For this review, take the finished solid that the model builds, in its own axes (mm). Give positions to 0.01 mm unless a question says otherwise; leave off trailing zeros. Write each loop counter-clockwise with the first axis right and the second up, starting at its lowest first coordinate (ties: lowest second). Pieces come first, ordered by that corner, then holes. Notation, with made-up numbers: M -12,-6 L 18,-6 A11 cw 18,13 Z; hole C -13,-8.75 d3. An arc over 180 degrees is marked long. Write item = value, one per line.
```python
from build123d import *

# Parameters (mm, degrees)
SKETCH_1_W            = 250
SKETCH_1_H            = 80
EXTRUDE_1_DEPTH       = 10
HOLE_WIZARD_9_0_9_1_D = 9
CHAMFER_1_SIZE        = 3
HOLE_WIZARD_M8_1_D    = 6.8
HOLE_WIZARD_M4_1_D    = 3.3


with BuildPart() as part:
    # 草图1 → 凸台-拉伸1 (new body)
    with BuildSketch(Plane.XY):
        with Locations((0, 40)):
            Rectangle(SKETCH_1_W, SKETCH_1_H)
    extrude(amount=EXTRUDE_1_DEPTH)

    # Ø9.0 (9) 直径孔1 (through all)
    with Locations(Plane.XY.offset(10)):
        with Locations((115, 20), (115, 60)):
            hole_wizard_9_0_9_1 = Hole(HOLE_WIZARD_9_0_9_1_D / 2)

    # 镜向1: Ø9.0 (9) 直径孔1 across plane
    add(hole_wizard_9_0_9_1.mirror(Plane(origin=(0, 0, 0), x_dir=(0, 0, 1), z_dir=(1, 0, 0))), mode=Mode.SUBTRACT)

    # 倒角1
    chamfer_1_edges = [part.edges().sort_by_distance(p)[0] for p in [
        (-125, 80, 5),
        (125, 80, 5),
        (125, 0, 5),
        (-125, 0, 5),
    ]]
    chamfer(chamfer_1_edges, length=CHAMFER_1_SIZE)

    # M8 螺纹孔1 (through all)
    with Locations(Plane.XY.offset(10)):
        with Locations((70.5, 60), (70.5, 20)):
            hole_wizard_m8_1 = Hole(HOLE_WIZARD_M8_1_D / 2)

    # 镜向2: M8 螺纹孔1 across plane
    add(hole_wizard_m8_1.mirror(Plane(origin=(0, 0, 0), x_dir=(0, 0, 1), z_dir=(1, 0, 0))), mode=Mode.SUBTRACT)

    # M4 螺纹孔1 (through all)
    with Locations(Plane.XY.offset(10)):
        with Locations((-94.121851999, 75), (-94.121851999, 5)):
            hole_wizard_m4_1 = Hole(HOLE_WIZARD_M4_1_D / 2)

    # 镜向3: M4 螺纹孔1 across plane
    add(hole_wizard_m4_1.mirror(Plane.ZY), mode=Mode.SUBTRACT)


solid = part.part
```
1. We need section C-C, the plane x = 115. Write out the cut boundary in (y, z), then the cut area to 3 significant figures.
Responses:
outline = M 0,0 L 15.5,0 L 15.5,10 L 0,10 Z; M 24.5,0 L 55.5,0 L 55.5,10 L 24.5,10 Z; M 64.5,0 L 80,0 L 80,10 L 64.5,10 Z
area = 620 mm2
2. We need section A-A, the plane x = -70.5. Write out the cut boundary in (y, z), then the cut area to 3 significant figures.
Responses:
outline = M 0,0 L 16.6,0 L 16.6,10 L 0,10 Z; M 23.4,0 L 56.6,0 L 56.6,10 L 23.4,10 Z; M 63.4,0 L 80,0 L 80,10 L 63.4,10 Z
area = 664 mm2
3. Insertion check: P1, Ø7, axis at x = -115, y = 20, coming from the -Z side. The pin has a flat end and moves straight along its axis. Give the tip position at first contact, or say it passes through.
Responses:
P1 = through
4. The part is to be moulded in two halves that separate along Y. For faces 1 (the face through (-125, 39, 5)), 2 (the face through (-2, 80, 5)), 3 (the face through (73.198, 17.931, 4.93)), say which applies: +Y half, -Y half, draft (parallel to the pull), parting line (faces both ways), or undercut.
Responses:
face_1 = draft
face_2 = +Y half
face_3 = undercut
5. For line 1 along Y through (x, z) = (-115, 5.75); line 2 along Y through (x, z) = (-70.5, 7); line 3 along X through (y, z) = (4.5, 9.5), list the stretches that pass through material, from the lowest coordinate up. Write a range as from..to.
Responses:
line_1 = 0..15.5, 24.5..55.5, 64.5..80
line_2 = 0..16.6, 23.4..56.6, 63.4..80
line_3 = -125..-95.69, -92.55..92.55, 95.69..125
6. We need section B-B, the plane y = 20. Write out the cut boundary in (x, z), then the cut area to 3 significant figures.
Responses:
outline = M -125,0 L -119.5,0 L -119.5,10 L -125,10 Z; M -110.5,0 L -73.9,0 L -73.9,10 L -110.5,10 Z; M -67.1,0 L 67.1,0 L 67.1,10 L -67.1,10 Z; M 73.9,0 L 110.5,0 L 110.5,10 L 73.9,10 Z; M 119.5,0 L 125,0 L 125,10 L 119.5,10 Z
area = 2,180 mm2
